Design review of the part built by this model. Coordinates are the model's own, in mm. A direction names the side the tool comes from. Coordinates: 2 decimals unless noted, no trailing zeros. Write each loop counter-clockwise with the first axis right and the second up, starting at its lowest first coordinate (ties: lowest second). Pieces come first, ordered by that corner, then holes.
Q1. Clearance check with a flat-ended pin moving along its axis: pin 1 Ø4 at (x, y) = (-49, -39) entering from -Z. State where the tip first meets the part, or that it passes through.
Q2. Add section B-B, the plane z = 105.5. Give the boundary of the cut face in (x, y), plus the area to 3 significant figures.
Q3. To check wall thickness, follow probe 1 along Y at (x, z) = (-30.5, 89.5); probe 2 along X at (y, z) = (-90, 261); probe 3 along X at (y, z) = (-137.5, 121). State the ranges of each line that lie inside material, in increasing order.
Q4. Machinability: for faces 5 (the face through (-49, -73, 136)), 6 (the face through (-23, 0, 136)), which of the approach directions +Z, -Z, +X, -X, +Y, -Y give a long, thin tool a straight path to every point of the face, cutting with its end or side? Answer none if there is none.
Q5. The part is to be moulded in two halves that separate along Y. For faces 1 (the face through (-23, -139, 136)), 2 (the face through (-14.79, -2.96, 218.22)), 3 (the face through (-24, -6, 136)), 4 (the face through (-24, -145, 136)), say which applies: +Y half, -Y half, draft (parallel to the pull), parting line (faces both ways), or undercut.
Q6. Add section C-C, the plane x = -17. Give the boundary of the cut face in (y, z), plus the area to 3 significant figures.
Q7. Add section D-D, the plane y = -117. Give the boundary of the cut face in (x, z), plus the area to 3 significant figures.
Q8. Add section A-A, the plane x = -33.5. Give the boundary of the cut face in (y, z), plus the area to 3 significant figures.
from build123d import *

# Parameters (mm, degrees)
EXTRUDE_1_DEPTH     = 275
CUT_EXTRUDE_1_DEPTH = 275


with BuildPart() as part:
    # 草图1 → 凸台-拉伸1 (new body)
    with BuildSketch(Plane.XY):
        with BuildLine():
            Line((0, 0), (-47, 0))
            ThreePointArc((-47, 0), (-52.656854249, -2.343145751), (-55, -8))
            Line((-55, -8), (-55, -137))
            ThreePointArc((-55, -137), (-52.656854249, -142.656854249), (-47, -145))
            Line((-47, -145), (0, -145))
            Line((0, -145), (0, -139))
            Line((0, -139), (-47, -139))
            ThreePointArc((-47, -139), (-48.414213562, -138.414213562), (-49, -137))
            Line((-49, -137), (-49, -8))
            ThreePointArc((-49, -8), (-48.414213562, -6.585786438), (-47, -6))
            Line((-47, -6), (0, -6))
            Line((0, -6), (0, 0))
        make_face()
    extrude(amount=EXTRUDE_1_DEPTH)

    # 草图2 → 切除-拉伸1 (cut)
    with BuildSketch(Plane(origin=(0, 0, 0), x_dir=(1, 0, 0), z_dir=(0, 1, 0))):
        Polygon((0, -163), (-30, -275), (0, -275), align=None)
    extrude(amount=-CUT_EXTRUDE_1_DEPTH, mode=Mode.SUBTRACT)


solid = part.part
Here are the results:
1. pin 1: stops at z = 0
2. outline: (-55, -137) arc R8 ccw to (-47, -145) - (0, -145) - (0, -139) - (-47, -139) arc R2 cw to (-49, -137) - (-49, -8) arc R2 cw to (-47, -6) - (0, -6) - (0, 0) - (-47, 0) arc R8 ccw to (-55, -8) - close
2. area: 1,430 mm2
3. probe 1: y = -145 to -139, -6 to 0
3. probe 2: x = -55 to -49
3. probe 3: x = -54.98 to -48.94
4. face 5: +Z, -Z, +X
4. face 6: +Z, -Z, +X, -X, +Y
5. face 1: undercut
5. face 2: draft
5. face 3: undercut
5. face 4: -Y half
6. outline: (-145, 0) - (-139, 0) - (-139, 226.47) - (-145, 226.47) - close; (-6, 0) - (0, 0) - (0, 226.47) - (-6, 226.47) - close
6. area: 2,720 mm2
7. outline: (-55, 0) - (-49, 0) - (-49, 275) - (-55, 275) - close
7. area: 1,650 mm2
8. outline: (-145, 0) - (-139, 0) - (-139, 275) - (-145, 275) - close; (-6, 0) - (0, 0) - (0, 275) - (-6, 275) - close
8. area: 3,300 mm2
